Verification items for the finished model (mm, model axes). Face numbers are marked on the shaded views. A direction names the side the tool comes from. Round coordinates to 2 decimals unless told otherwise and drop trailing zeros. Loops run counter-clockwise (first coordinate to the right, second up) from the corner with the lowest first, then second, coordinate; pieces in that order, holes last. Notation, with made-up numbers: (87.25, 41.5) -> (138.25, 41.5) arc R28 cw to (138.25, 76.5) -> close; hole circle Ø2 at (58.5, -9.5). An arc over 180 degrees is marked (long way). Write item = value, one per line. Start each with the question number.
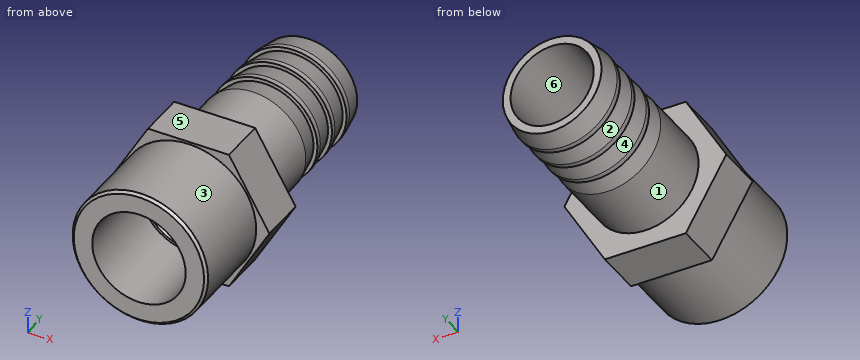
```python
from build123d import *

# Parameters (mm, degrees)
EXTRUDE_1_DEPTH     = 9
SKETCH_3_R          = 13.05
EXTRUDE_2_DEPTH     = 17
CUT_EXTRUDE_1_REACH = 63.557
SKETCH_4_R          = 8
SKETCH_5_R          = 9
CUT_EXTRUDE_2_DEPTH = 17
CHAMFER_1_SIZE      = 0.5
CHAMFER_2_SIZE      = 0.5


with BuildPart() as part:
    # 草图1 → 旋转1 (revolve)
    with BuildSketch(Plane.XY, mode=Mode.PRIVATE) as revolve_1_sk:
        Polygon((-10.25, 13), (-9.5, 17), (-10.25, 17), (-10.25, 18), (-9.5, 22), (-10.25, 22), (-10.25, 23), (-9.5, 27), (-10.25, 27), (-10.25, 28), (-9.5, 32), (0, 32), (0, 0), (-10.25, 0), align=None)
    revolve(revolve_1_sk.sketch.rotate(Axis((0, 0, 0), (0, 1, 0)), 180), axis=Axis((0, 0, 0), (0, 1, 0)))

    # 草图2 → 凸台-拉伸1 (add)
    with BuildSketch(Plane.XZ):
        Polygon((15.588457268, 0), (7.794228634, 13.5), (-7.794228634, 13.5), (-15.588457268, 0), (-7.794228634, -13.5), (7.794228634, -13.5), align=None)
    extrude(amount=EXTRUDE_1_DEPTH)

    # 草图3 → 凸台-拉伸2 (add)
    with BuildSketch(Plane.XZ.offset(9)):
        Circle(SKETCH_3_R)
    extrude(amount=EXTRUDE_2_DEPTH)

    # 草图4 → 切除-拉伸1 (cut, up to next)
    with BuildSketch(Plane(origin=(0, 32, 0), x_dir=(1, 0, 0), z_dir=(0, 1, 0)), mode=Mode.PRIVATE) as cut_extrude_1_sk1:
        with Locations(Location((0, 0, 0), (0, 0, 180))):
            Circle(SKETCH_4_R)
    cut_extrude_1_tool1 = extrude(cut_extrude_1_sk1.sketch, amount=-CUT_EXTRUDE_1_REACH, mode=Mode.PRIVATE) & part.part
    add(cut_extrude_1_tool1.solids().sort_by_distance((0, 32, 0))[0], mode=Mode.SUBTRACT)

    # 草图5 → 切除-拉伸2 (cut)
    with BuildSketch(Plane.XZ.offset(26)):
        Circle(SKETCH_5_R)
    extrude(amount=-CUT_EXTRUDE_2_DEPTH, mode=Mode.SUBTRACT)

    # 倒角1
    chamfer_1_edges = [part.edges().sort_by_distance(p)[0] for p in [
        (-13.05, -26, 0),
    ]]
    chamfer(chamfer_1_edges, length=CHAMFER_1_SIZE)

    # 倒角2
    chamfer_2_edges = [part.edges().sort_by_distance(p)[0] for p in [
        (8, -9, 0),
    ]]
    chamfer(chamfer_2_edges, length=CHAMFER_2_SIZE)


solid = part.part
```
(1) Section check C-C on y = -21. Enter the section's corners in (x, z).
(2) Depth check by flat-ended pin: pin 1 Ø5 at (y, z) = (0.5, 8.5) entering from +X; pin 2 Ø2 at (y, z) = (8.5, 6) entering from +X; pin 3 Ø8 at (x, y) = (-12, 16.5) entering from -Z. Enter the tip coordinate at first touch or a pass-through.
(3) Section check B-B on y = 6. Enter the section's corners in (x, z), then the cut area to 3 significant figures.
(4) Access from +Z, -Z, +X, -X, +Y, -Y to the whole of each face (thin tool, end or side, straight path). Record for the marked faces 1, 2 and 3.
(5) Section check A-A on y = -6. Enter the section's corners in (x, z), then the cut area to 3 significant figures.
(6) Scan lines: line 1 (Z direction, x = 0, y = -15.75); line 2 (X direction, y = -23, z = 0.5); line 3 (Z direction, x = 0, y = 11.5). Record each from-to range of solid material in increasing order. Write a range as [from, to].
(7) Draft check along Z on the marked faces 4, 5 and 6. Enter one of: +Z half, -Z half, draft (parallel to the pull), parting line (faces both ways), or undercut.
Computed values:
q1.outline = circle Ø26.1 at (0, 0); hole circle Ø18 at (0, 0)
q2.pin_1 = 12.1
q2.pin_2 = 8.95
q2.pin_3 = -6.37
q3.outline = circle Ø20.5 at (0, 0); hole circle Ø16 at (0, 0)
q3.area = 129 mm²
q4.face_1 = +Y
q4.face_2 = none
q4.face_3 = -Y
q5.outline = (-15.59, 0) -> (-7.79, -13.5) -> (7.79, -13.5) -> (15.59, 0) -> (7.79, 13.5) -> (-7.79, 13.5) -> close; hole circle Ø16 at (0, 0)
q5.area = 430 mm²
q6.line_1 = [-13.05, -9], [9, 13.05]
q6.line_2 = [-13.04, -8.99], [8.99, 13.04]
q6.line_3 = [-10.25, -8], [8, 10.25]
q7.face_4 = parting line
q7.face_5 = +Z half
q7.face_6 = undercut
